from build123d import *

# Parameters (mm, degrees)
BOSS_EXTRUDE1_DEPTH = 30
CUT_EXTRUDE1_START  = -5
CUT_EXTRUDE1_DEPTH  = 5
BOSS_EXTRUDE2_DEPTH = 1
SKETCH4_W           = 5
SKETCH4_H           = 2
BOSS_EXTRUDE3_DEPTH = 20.16339138
SKETCH5_W           = 5
SKETCH5_H           = 10.599022434
BOSS_EXTRUDE4_DEPTH = 1.154700538
CUT_EXTRUDE2_DEPTH  = 5
BOSS_EXTRUDE5_DEPTH = 1
SKETCH8_W           = 5
SKETCH8_H           = 2
BOSS_EXTRUDE6_DEPTH = 20.16339138
SKETCH9_W           = 5
SKETCH9_H           = 10.599022434
BOSS_EXTRUDE7_DEPTH = 1.154700538
BOSS_EXTRUDE8_DEPTH = 2
DRAFT1_ANGLE        = 30
DRAFT2_ANGLE        = 30
FILLET1_R           = 2
FILLET2_R           = 4


with BuildPart() as part:
    # Sketch1 → Boss-Extrude1 (new body)
    with BuildSketch(Plane(origin=(-30, 0, 0), x_dir=(0, -1, 0), z_dir=(-1, 0, 0))):
        with BuildLine():
            Line((0, -1), (0, -2))
            ThreePointArc((0, -2), (1, -3), (2, -2))
            Line((2, -2), (2, -1))
            ThreePointArc((2, -1), (1, 0), (0, -1))
        make_face()
    extrude(amount=-BOSS_EXTRUDE1_DEPTH)

    # Sketch2 → Cut-Extrude1 (cut)
    with BuildSketch(Plane(origin=(0, 0, 0), x_dir=(0, 0, -1), z_dir=(1, 0, 0)).offset(CUT_EXTRUDE1_START)):
        with BuildLine():
            Line((2, 0), (2, -2))
            ThreePointArc((2, -2), (3, -1), (2, 0))
        make_face()
    extrude(amount=CUT_EXTRUDE1_DEPTH, mode=Mode.SUBTRACT)

    # Sketch3 → Boss-Extrude2 (add)
    with BuildSketch(Plane(origin=(0, 0, -2), x_dir=(-1, 0, 0), z_dir=(0, 0, -1))):
        Polygon((5, -2), (0, -2), (0, 0), (5, 0), (5, -1), align=None)
    extrude(amount=BOSS_EXTRUDE2_DEPTH)

    # Sketch4 → Boss-Extrude3 (add)
    with BuildSketch(Plane(origin=(0, 0, -3), x_dir=(-1, 0, 0), z_dir=(0, 0, -1))):
        with Locations((2.5, -1)):
            Rectangle(SKETCH4_W, SKETCH4_H)
    extrude(amount=BOSS_EXTRUDE3_DEPTH)

    # Sketch5 → Boss-Extrude4 (add)
    with BuildSketch(Plane(origin=(0, 0, -23.16339138), x_dir=(-1, 0, 0), z_dir=(0, 0, -1))):
        with Locations((2.5, -5.299511217)):
            Rectangle(SKETCH5_W, SKETCH5_H)
    extrude(amount=BOSS_EXTRUDE4_DEPTH)

    # Sketch6 → Cut-Extrude2 (cut)
    with BuildSketch(Plane.ZY.offset(30)):
        with BuildLine():
            Line((-2, -2), (-2, 0))
            ThreePointArc((-2, 0), (-3, -1), (-2, -2))
        make_face()
    extrude(amount=-CUT_EXTRUDE2_DEPTH, mode=Mode.SUBTRACT)

    # Sketch7 → Boss-Extrude5 (add)
    with BuildSketch(Plane(origin=(0, 0, -2), x_dir=(-1, 0, 0), z_dir=(0, 0, -1))):
        Polygon((30, -2), (25, -2), (25, -1), (25, 0), (30, 0), align=None)
    extrude(amount=BOSS_EXTRUDE5_DEPTH)

    # Sketch8 → Boss-Extrude6 (add)
    with BuildSketch(Plane(origin=(0, 0, -3), x_dir=(-1, 0, 0), z_dir=(0, 0, -1))):
        with Locations((27.5, -1)):
            Rectangle(SKETCH8_W, SKETCH8_H)
    extrude(amount=BOSS_EXTRUDE6_DEPTH)

    # Sketch9 → Boss-Extrude7 (add)
    with BuildSketch(Plane(origin=(0, 0, -23.16339138), x_dir=(-1, 0, 0), z_dir=(0, 0, -1))):
        with Locations((27.5, -5.299511217)):
            Rectangle(SKETCH9_W, SKETCH9_H)
    extrude(amount=BOSS_EXTRUDE7_DEPTH)

    # Sketch10 → Boss-Extrude8 (add)
    with BuildSketch(Plane.XZ.offset(10.599022434)):
        Polygon((0, -23.16339138), (0, -37.525669468), (-30, -37.525669468), (-30, -23.16339138), (-25, -23.16339138), (-25, -32.525669468), (-5, -32.525669468), (-5, -23.16339138), align=None)
    extrude(amount=BOSS_EXTRUDE8_DEPTH)

    # Draft1
    draft1_faces = [part.faces().sort_by_distance(p)[0] for p in [
        (-2.5, -5.299511217, -24.318091918),
        (-27.5, -5.299511217, -24.318091918),
    ]]
    draft(draft1_faces, Plane(origin=(0, 0, -1), x_dir=(0, 0, 1), z_dir=(0, 1, 0)), DRAFT1_ANGLE)

    # Draft2
    draft2_faces = [part.faces().sort_by_distance(p)[0] for p in [
        (-27.5, -7.299511217, -23.16339138),
        (-2.5, -7.299511217, -23.16339138),
    ]]
    draft(draft2_faces, Plane(origin=(0, -2, -2), x_dir=(0, 0, -1), z_dir=(0, -1, 0)), DRAFT2_ANGLE)

    # Fillet1
    fillet1_edges = [part.edges().sort_by_distance(p)[0] for p in [
        (-27.5, -10.599022434, -30.437440374),
        (-2.5, -2, -23.16339138),
        (-2.5, -10.599022434, -30.437440374),
        (-27.5, -2, -23.16339138),
    ]]
    fillet(fillet1_edges, radius=FILLET1_R)

    # Fillet2
    fillet2_edges = [part.edges().sort_by_distance(p)[0] for p in [
        (-27.5, 0, -24.318091918),
        (-2.5, -12.599022434, -29.282739835),
        (-27.5, -12.599022434, -29.282739835),
        (-2.5, 0, -24.318091918),
    ]]
    fillet(fillet2_edges, radius=FILLET2_R)


solid = part.part
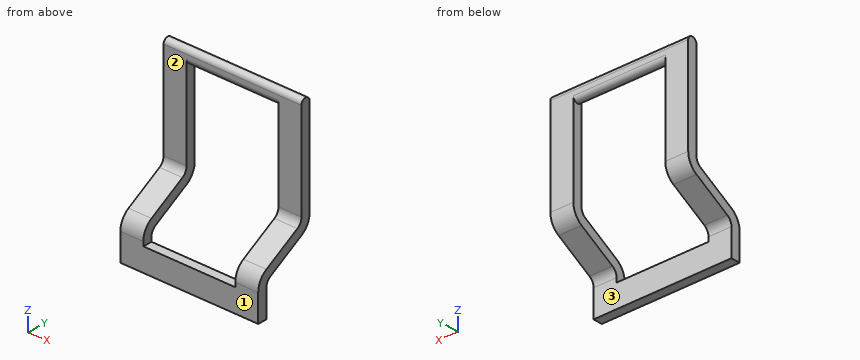
The listing builds one solid part. Answer for the finished solid, in the listing's coordinates (mm). Face numbers are marked on the shaded views. A direction names the side the tool comes from. Give positions to 0.01 mm unless a question says otherwise; leave off trailing zeros. Write each loop counter-clockwise with the first axis right and the second up, starting at its lowest first coordinate (ties: lowest second). Pieces come first, ordered by that corner, then holes. Notation, with made-up numbers: (30.25, 88) -> (76.25, 88) arc R15 cw to (76.25, 95) -> close; hole circle Ø2 at (64.5, 9.25). An arc over 180 degrees is marked (long way). One line per question, with ' | ' between items. Start each with the question number.
1. Section B-B (x = -18.5) is taken. Determine the outline of the cut face in (y, z), plus the area to 3 significant figures.
2. For the marked faces 1, 2 and 3, determine the directions among +Z, -Z, +X, -X, +Y, -Y from which every point of the face is accessible in a straight line to the end or side of a thin tool.
3. Given pin 1 Ø3 at (x, z) = (-8, -34) entering from +Y; pin 2 Ø2 at (x, y) = (-19, -11) entering from +Z, each flat-ended and moving along its own axis, determine where each tip first touches the part or whether it passes through.
4. Section C-C (x = -3) is taken. Determine the outline of the cut face in (y, z).
5. Find the intervals of material crossed by probe 1 along Y at (x, z) = (-1.5, -6); probe 2 along Z at (x, y) = (-18.5, -11.75); probe 3 along Z at (x, y) = (-12.5, -1), in increasing order.
6. Section A-A (z = -15) is taken. Determine the outline of the cut face in (x, y).
7. Section D-D (y = -1) is taken. Determine the outline of the cut face in (x, z), plus the area to 3 significant figures.
Response values:
1) outline: (-12.6, -37.53) -> (-10.6, -37.53) -> (-10.6, -32.53) -> (-12.6, -32.53) -> close; (-2, -2) arc R1 ccw to (0, -2) -> (0, -1) arc R1 ccw to (-2, -1) -> close | area: 15.1 mm2
2) face 1: +Z, -Z, +X, -X, -Y | face 2: +Z, +X, -X, -Y | face 3: -Z, +X, -X, +Y
3) pin 1: y = -10.6 | pin 2: z = -32.53
4) outline: (-12.6, -37.53) -> (-10.6, -37.53) -> (-10.6, -31.59) arc R2 cw to (-9.6, -29.86) -> (-2, -25.47) arc R4 ccw to (0, -22.01) -> (0, -1) arc R1 ccw to (-2, -1) -> (-2, -22.01) arc R2 cw to (-3, -23.74) -> (-10.6, -28.13) arc R4 ccw to (-12.6, -31.59) -> close
5) probe 1: -2 to 0 | probe 2: -37.53 to -32.53 | probe 3: -3 to 0
6) outline: (-30, -2) -> (-25, -2) -> (-25, 0) -> (-30, 0) -> close; (-5, -2) -> (0, -2) -> (0, 0) -> (-5, 0) -> close
7) outline: (-30, -24.65) -> (-25, -24.65) -> (-25, -3) -> (-5, -3) -> (-5, -24.65) -> (0, -24.65) -> (0, 0) -> (-30, 0) -> close | area: 307 mm2
